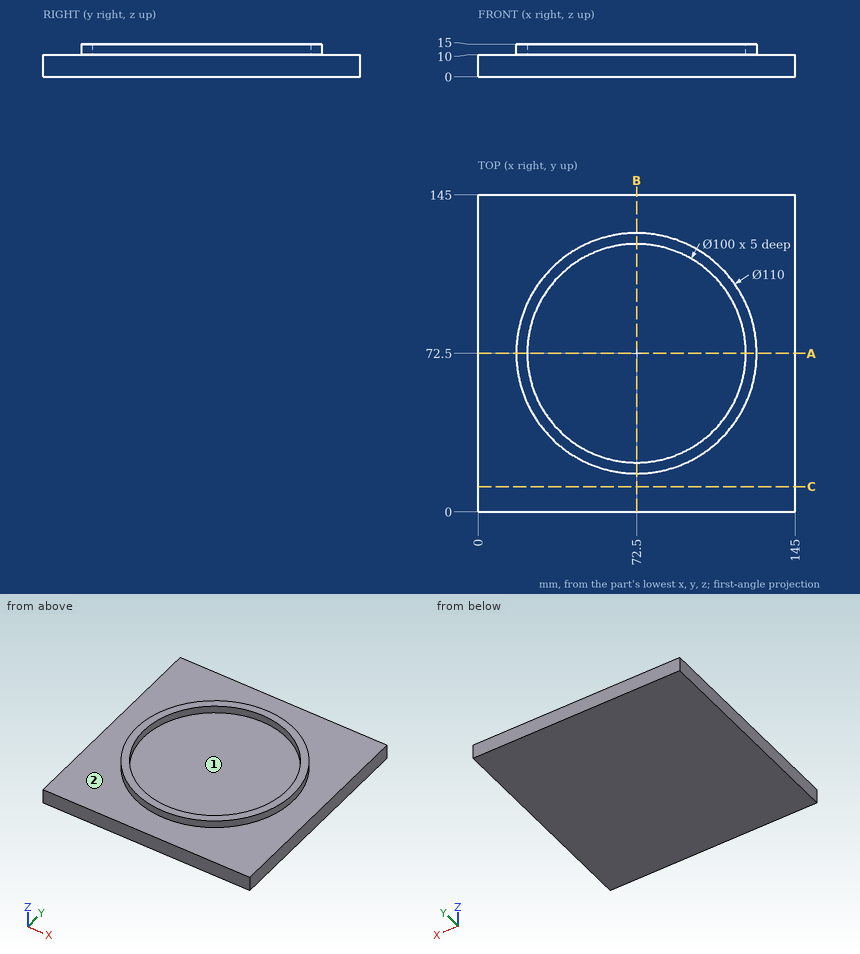
Part print with two shaded views. Sizes in mm from the minimum x, y, z corner. Round coordinates to 2 decimals unless told otherwise and drop trailing zeros. Order: outer loops, then holes, each group sorted by start corner. A loop starts at its lowest first (then second) coordinate and runs counter-clockwise, first axis right, second up.
(1) Band-saw the part on A-A (y = 72.5). List the corners of the cut face in (x, z), then the cut area to 3 significant figures.
(2) Drill centre lines: line 1 (Y direction, x = 72.5, z = 11.45); line 2 (Z direction, x = 121, y = 39.5); line 3 (Y direction, x = 64, z = 12.5). Where is each one in solid material? Low to high.
(3) Band-saw the part on C-C (y = 11.5). List the corners of the cut face in (x, z), then the cut area to 3 significant figures.
(4) Pull direction X, two halves, no side cores. Call the marked faces 1 and 2: released by +X, released by -X, zero draft, split by the parting line, or undercut.
(5) Pin check, flat tip, straight feed: pin 1 (1.5 mm diameter, centred on x = 67.5, y = 65.5, fed in from +Z). Stop position of the tip, or through.
Verdict:
1. outline: (0, 0) - (145, 0) - (145, 10) - (127.5, 10) - (127.5, 15) - (122.5, 15) - (122.5, 10) - (22.5, 10) - (22.5, 15) - (17.5, 15) - (17.5, 10) - (0, 10) - close
1. area: 1,500 mm2
2. line 1: y = 17.5 to 22.5, 122.5 to 127.5
2. line 2: z = 0 to 10
2. line 3: y = 18.16 to 23.23, 121.77 to 126.84
3. outline: (0, 0) - (145, 0) - (145, 10) - (0, 10) - close
3. area: 1,450 mm2
4. face 1: undercut
4. face 2: zero draft
5. pin 1: stops at z = 10
